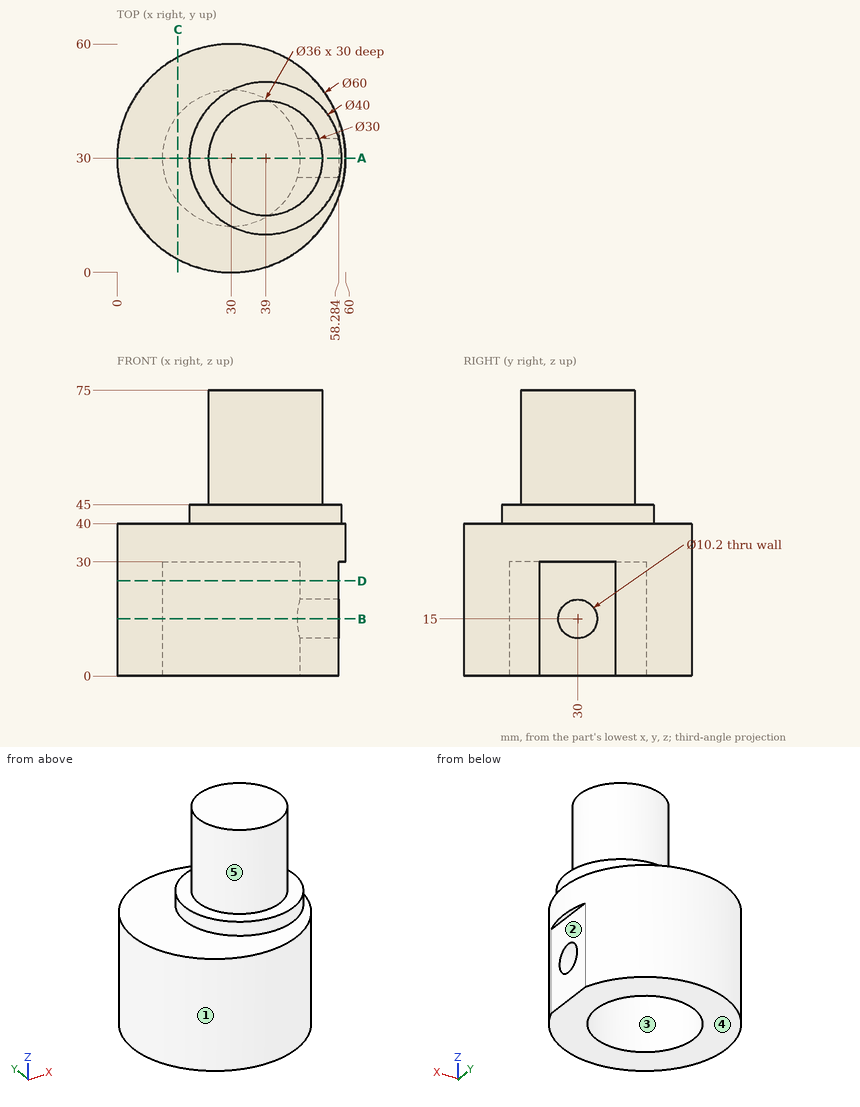
Study the drawing (mm; zero at the part's minimum x, y, z) and answer. A direction names the side the tool comes from. Coordinates: 2 decimals unless noted, no trailing zeros. Loops run counter-clockwise (first coordinate to the right, second up) from the corner with the lowest first, then second, coordinate; pieces in that order, holes last. Notation, with made-up numbers: M 23,1 L 57,1 A17 ccw 57,19 Z; hole C 24,86.5 d4. An arc over 180 degrees is marked long. Answer in a Markdown table with one row per item. Add a question column.
1. The mould has two halves that part along X. Classify the marked faces 1, 2 and 3: pulls with the +X half, pulls with the -X half, needs draft (parallel to the pull), parting line crosses it, or undercut.
2. Consider L1, parallel to Y at x = 30, z = 11; L2, parallel to Y at x = 54, z = 15; L3, parallel to Z at x = 54.75, y = 30. Determine where each line is inside the solid, lowest interval first.
3. Find section B-B, the plane z = 15. Write down the section's boundary in (x, y), then the cut area to 3 significant figures.
4. Find section D-D, the plane z = 25. Write down the section's boundary in (x, y), then the cut area to 3 significant figures.
5. Flat-ended cylindrical pins translate along their axes: P1, Ø18, axis at x = 34, y = 32, coming from the -Z side; P2, Ø1.5, axis at x = 22, z = 40, coming from the +Y side; P3, Ø1, axis at y = 43, z = 11.5, coming from the -X side. Find the tip coordinate at first contact, or state that the pin passes through.
6. A tool of negligible diameter and unlimited length cuts with its end or side. For the marked faces 4 and 5, from which of +Z, -Z, +X, -X, +Y, -Y can it reach the whole face along a straight path? Write none if from no direction.
7. Find section A-A, the plane y = 30. Write down the section's boundary in (x, z).
8. Find section C-C, the plane x = 16. Write down the section's boundary in (y, z).
Reported:
| question | item | result |
|---|---|---|
| 1 | face 1 | parting line crosses it |
| 1 | face 2 | pulls with the +X half |
| 1 | face 3 | undercut |
| 2 | L1 | y = 0 to 12, 48 to 60 |
| 2 | L2 | y = 12 to 24.9, 35.1 to 48 |
| 2 | L3 | z = 0 to 9.9, 20.1 to 45 |
| 3 | outline | M 47.26,24.9 A18 cw long 47.26,35.1 L 58.28,35.1 L 58.28,40 A30 ccw long 58.28,20 L 58.28,24.9 Z |
| 3 | area | 1,680 mm^2 |
| 4 | outline | M 58.28,20 L 58.28,40 A30 ccw long Z; hole C 30,30 d36 |
| 4 | area | 1,790 mm^2 |
| 5 | P1 | stops at z = 30 |
| 5 | P2 | stops at y = 59.11 |
| 5 | P3 | stops at x = 2.73 |
| 6 | face 4 | -Z, +X, -X, +Y, -Y |
| 6 | face 5 | +Z |
| 7 | outline | M 0,0 L 12,0 L 12,30 L 48,30 L 48,20.1 L 58.28,20.1 L 58.28,30 L 60,30 L 60,40 L 59,40 L 59,45 L 54,45 L 54,75 L 24,75 L 24,45 L 19,45 L 19,40 L 0,40 Z; M 48,0 L 58.28,0 L 58.28,9.9 L 48,9.9 Z |
| 8 | outline | M 3.47,0 L 18.69,0 L 18.69,30 L 41.31,30 L 41.31,0 L 56.53,0 L 56.53,40 L 3.47,40 Z |
